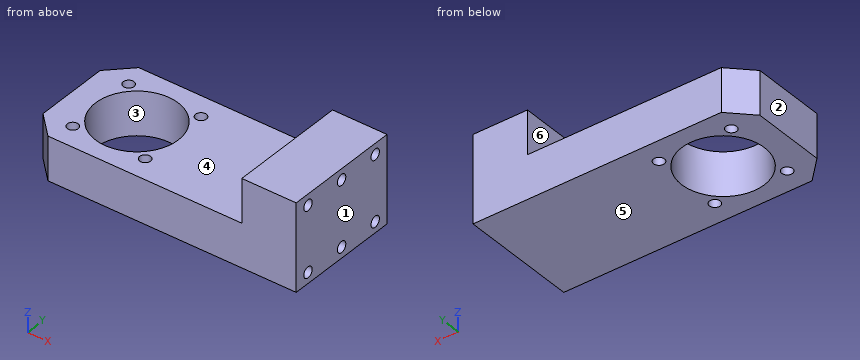
from build123d import *

# Parameters (mm, degrees)
SKETCH1_W             = 124
SKETCH1_H             = 54
BOSS_EXTRUDE1_DEPTH   = 20
CHAMFER1_SIZE         = 10
SKETCH2_R             = 19
CUT_EXTRUDE1_DEPTH    = 20
M6_TAPPED_HOLE1_D     = 5
CIRPATTERN1_COUNT     = 4
SKETCH7_W             = 25
SKETCH7_H             = 54
BOSS_EXTRUDE2_DEPTH   = 20
M6_TAPPED_HOLE2_D     = 5
M6_TAPPED_HOLE2_DEPTH = 15
M6_TAPPED_HOLE2_TIP   = 1.502151548


with BuildPart() as part:
    # Sketch1 → Boss-Extrude1 (new body)
    with BuildSketch(Plane.XY):
        with Locations((62, 27)):
            Rectangle(SKETCH1_W, SKETCH1_H)
    extrude(amount=BOSS_EXTRUDE1_DEPTH)

    # Chamfer1
    chamfer1_edges = [part.edges().sort_by_distance(p)[0] for p in [
        (0, 54, 10),
        (0, 0, 10),
    ]]
    chamfer(chamfer1_edges, length=CHAMFER1_SIZE)

    # Sketch2 → Cut-Extrude1 (cut)
    with BuildSketch(Plane.XY.offset(20)):
        with Locations((30, 27)):
            Circle(SKETCH2_R)
    extrude(amount=-CUT_EXTRUDE1_DEPTH, mode=Mode.SUBTRACT)

    # M6 Tapped Hole1 (through all)
    with Locations(Plane.XY.offset(20)):
        with Locations((46.617009358, 43.617009358)):
            m6_tapped_hole1 = Hole(M6_TAPPED_HOLE1_D / 2)

    # CirPattern1: M6 Tapped Hole1 ×4 about axis
    cirpattern1_axis = Axis((30, 27, 0), (0, 0, 1))
    for i in range(1, CIRPATTERN1_COUNT):
        add(m6_tapped_hole1.rotate(cirpattern1_axis, i * 360 / CIRPATTERN1_COUNT), mode=Mode.SUBTRACT)

    # Sketch7 → Boss-Extrude2 (add)
    with BuildSketch(Plane.XY.offset(20)):
        with Locations((111.5, 27)):
            Rectangle(SKETCH7_W, SKETCH7_H)
    extrude(amount=BOSS_EXTRUDE2_DEPTH)

    # M6 Tapped Hole2
    with Locations(Plane(origin=(124, 0, 0), x_dir=(0, 0, -1), z_dir=(1, 0, 0))):
        with Locations((-35, 47), (-5, 47), (-35, 7), (-5, 7), (-35, 27), (-5, 27)):
            Hole(M6_TAPPED_HOLE2_D / 2, depth=M6_TAPPED_HOLE2_DEPTH)
            with Locations((0, 0, -(M6_TAPPED_HOLE2_DEPTH + M6_TAPPED_HOLE2_TIP / 2))):  # 118° drill point
                Cone(0, M6_TAPPED_HOLE2_D / 2, M6_TAPPED_HOLE2_TIP, mode=Mode.SUBTRACT)


solid = part.part
For this review, take the finished solid that the model builds, in its own axes (mm). Face numbers are marked on the shaded views. A direction names the side the tool comes from. Round coordinates to 2 decimals unless told otherwise and drop trailing zeros. Loops run counter-clockwise (first coordinate to the right, second up) from the corner with the lowest first, then second, coordinate; pieces in that order, holes last. Notation, with made-up numbers: (57.5, 53.25) - (65.5, 53.25) arc R8 ccw to (65.5, 57.25) - close; hole circle Ø5 at (-17, 19). An arc over 180 degrees is marked (long way). One line per question, with ' | ' between items.
Q1. Take a section at D-D (y = 3). Give the boundary of the cut face in (x, z), and give its area (3 significant figures).
Taken from the geometry:
outline: (7, 0) - (124, 0) - (124, 40) - (99, 40) - (99, 20) - (7, 20) - close | area: 2,840 mm²
Q2. Tool access review of the marked faces 5 and 6: name each direction out of +Z, -Z, +X, -X, +Y, -Y from which nothing blocks a thin tool from reaching the whole face with its end or side.
Taken from the geometry:
face 5: -Z, +X, -X, +Y, -Y | face 6: +Z, -X, +Y, -Y
Q3. The part is to be moulded in two halves that separate along X. For the marked faces 1, 2, 3 and 4, say which applies: released by +X, released by -X, zero draft, split by the parting line, or undercut.
Taken from the geometry:
face 1: released by +X | face 2: released by -X | face 3: undercut | face 4: zero draft
Q4. Take a section at C-C (z = 9). Give the boundary of the cut face in (x, y).
Taken from the geometry:
outline: (0, 10) - (10, 0) - (124, 0) - (124, 54) - (10, 54) - (0, 44) - close; hole circle Ø5 at (13.38, 10.38); hole circle Ø5 at (13.38, 43.62); hole circle Ø38 at (30, 27); hole circle Ø5 at (46.62, 10.38); hole circle Ø5 at (46.62, 43.62)
Q5. For line 1 along Y through (x, z) = (114.75, 35); line 2 along Z through (x, y) = (119.25, 47); line 3 along Z through (x, y) = (60.5, 12), list the stretches that pass through material, from the lowest coordinate up. Write a range as [from, to].
Taken from the geometry:
line 1: y = [0, 4.5], [9.5, 24.5], [29.5, 44.5], [49.5, 54] | line 2: z = [0, 2.5], [7.5, 32.5], [37.5, 40] | line 3: z = [0, 20]
Q6. Take a section at A-A (x = 30). Give the boundary of the cut face in (y, z), and give its area (3 significant figures).
Taken from the geometry:
outline: (0, 0) - (8, 0) - (8, 20) - (0, 20) - close; (46, 0) - (54, 0) - (54, 20) - (46, 20) - close | area: 320 mm²
Q7. Take a section at B-B (y = 19). Give the boundary of the cut face in (x, z), and give its area (3 significant figures).
Taken from the geometry:
outline: (0, 0) - (12.77, 0) - (12.77, 20) - (0, 20) - close; (47.23, 0) - (124, 0) - (124, 40) - (99, 40) - (99, 20) - (47.23, 20) - close | area: 2,290 mm²
Q8. For pin 1 (6.5 mm diameter, centred on y = 27, z = 35, fed in from +X); pin 2 (2 mm diameter, centred on y = 22, z = 32.5, fed in from -X); pin 3 (16 mm diameter, centred on x = 60.5, y = 33, fed in from +Z); pin 4 (4 mm diameter, centred on y = 7, z = 5, fed in from -X), all flat-tipped, find the tip position at first contact; note any pin that passes through.
Taken from the geometry:
pin 1: stops at x = 124 | pin 2: stops at x = 99 | pin 3: stops at z = 20 | pin 4: stops at x = 1
